from build123d import *


with BuildPart() as part:
    # Sketch1 → Revolve1 (revolve)
    with BuildSketch(Plane.XY, mode=Mode.PRIVATE) as revolve1_sk:
        Polygon((55, 0), (55, 33), (48.5, 33), (48.5, 217), (55, 217), (55, 250), (62.5, 250), (62.5, 228), (63.5, 228), (63.5, 33), (62.5, 33), (62.5, 0), align=None)
    revolve(revolve1_sk.sketch.rotate(Axis((0, 0, 0), (0, 1, 0)), 90), axis=Axis((0, 0, 0), (0, 1, 0)))


solid = part.part
Work out the finished part from the listing and answer in its coordinate system (mm). A direction names the side the tool comes from. Give positions to 0.01 mm unless a question says otherwise; leave off trailing zeros. Write each loop counter-clockwise with the first axis right and the second up, starting at its lowest first coordinate (ties: lowest second). Pieces come first, ordered by that corner, then holes. Notation, with made-up numbers: (-23.5, 83) - (26.5, 83) arc R20 cw to (26.5, 95) - close; hole circle Ø10 at (50, -9.75). An arc over 180 degrees is marked (long way). One line per item, written item: value. Start each with the question number.
1. Find section A-A (x = 14.5). Write down the section's boundary in (y, z), then the cut area to 3 significant figures.
2. For faces 5 (the flat face through (42, 33, -47)), 6 (the flat face through (55.3, 250, -0.3)), 7 (the flat face through (49, 217, 0)), determine the directions among +Z, -Z, +X, -X, +Y, -Y from which every point of the face is accessible in a straight line to the end or side of a thin tool.
3. For a pull along Z with two mould halves and no side action, classify faces 1 (the cylindrical face through (48.794, 233.731, -25.379)), 2 (the cylindrical face through (-2.75, 238.85, 62.44)), 3 (the cylindrical face through (43.028, 126.288, -22.38)), 4 (the flat face through (42, 228, 47)) as +Z half, -Z half, draft (parallel to the pull), parting line (faces both ways), or undercut.
4. Find section B-B (z = 0). Write down the section's boundary in (x, y), then the cut area to 3 significant figures.
5. Consider probe 1 along X at (y, z) = (233, 0); probe 2 along X at (y, z) = (75, 0); probe 3 along Z at (x, y) = (-48, 17). Determine where each line is inside the solid, lowest interval first.
6. Given pin 1 (3 mm diameter, centred on x = -30, y = 109.5, fed in from -Z); pin 2 (12 mm diameter, centred on x = 15.5, y = 150, fed in from +Z); pin 3 (8 mm diameter, centred on y = 60, z = 24, fed in from +X), each flat-ended and moving along its own axis, determine where each tip first touches the part or whether it passes through.
7. Find section C-C (y = 102.5). Write down the section's boundary in (x, z), then the cut area to 3 significant figures.
Geometry results:
1. outline: (0, -60.79) - (33, -60.79) - (33, -61.82) - (228, -61.82) - (228, -60.79) - (250, -60.79) - (250, -53.05) - (217, -53.05) - (217, -46.28) - (33, -46.28) - (33, -53.05) - (0, -53.05) - close; (0, 53.05) - (33, 53.05) - (33, 46.28) - (217, 46.28) - (217, 53.05) - (250, 53.05) - (250, 60.79) - (228, 60.79) - (228, 61.82) - (33, 61.82) - (33, 60.79) - (0, 60.79) - close
1. area: 6,760 mm2
2. face 5: -Y
2. face 6: +Z, -Z, +X, -X, +Y
2. face 7: +Y
3. face 1: undercut
3. face 2: parting line
3. face 3: undercut
3. face 4: draft
4. outline: (-63.5, 33) - (-62.5, 33) - (-62.5, 0) - (-55, 0) - (-55, 33) - (-48.5, 33) - (-48.5, 217) - (-55, 217) - (-55, 250) - (-62.5, 250) - (-62.5, 228) - (-63.5, 228) - close; (48.5, 33) - (55, 33) - (55, 0) - (62.5, 0) - (62.5, 33) - (63.5, 33) - (63.5, 228) - (62.5, 228) - (62.5, 250) - (55, 250) - (55, 217) - (48.5, 217) - close
4. area: 6,530 mm2
5. probe 1: -62.5 to -55, 55 to 62.5
5. probe 2: -63.5 to -48.5, 48.5 to 63.5
5. probe 3: -40.03 to -26.85, 26.85 to 40.03
6. pin 1: z = -56.75
6. pin 2: z = 62.79
6. pin 3: x = 60.27
7. outline: circle Ø127 at (0, 0); hole circle Ø97 at (0, 0)
7. area: 5,280 mm2
